Can you work these out from the model? Positions are in its coordinate system, mm. A direction names the side the tool comes from. Give positions to 0.01 mm unless a question says otherwise; leave off trailing zeros. Order: outer loops, then holes, each group sorted by start corner. A loop starts at its lowest first (then second) coordinate and runs counter-clockwise, first axis right, second up. Notation, with made-up numbers: (10, 43.25) - (61, 43.25) arc R8 ccw to (61, 50.25) - close; hole circle Ø11 at (0.25, -20.5). An arc over 180 degrees is marked (long way). Answer as CSV lines item,"result".
```python
from build123d import *

# Parameters (mm, degrees)
SKETCH1_R           = 25
BOSS_EXTRUDE1_DEPTH = 42
CHAMFER1_SIZE       = 1.5


with BuildPart() as part:
    # Sketch1 → Boss-Extrude1 (new body)
    with BuildSketch(Plane(origin=(0, 0, 0), x_dir=(1, 0, 0), z_dir=(0, 1, 0))):
        with Locations(Location((0, 0, 0), (0, 0, 90))):
            Circle(SKETCH1_R)
        with BuildLine():
            ThreePointArc((10, 0), (8.062257748, -5.916079783), (3, -9.539392014))
            Line((3, -9.539392014), (3, -12.8))
            Line((3, -12.8), (-3, -12.8))
            Line((-3, -12.8), (-3, -9.539392014))
            ThreePointArc((-3, -9.539392014), (-5.916079783, 8.062257748), (10, 0))
        make_face(mode=Mode.SUBTRACT)
    extrude(amount=BOSS_EXTRUDE1_DEPTH)

    # Chamfer1
    chamfer1_edges = [part.edges().sort_by_distance(p)[0] for p in [
        (-5.916079783, 42, -8.062257748),
        (-5.916079783, 0, -8.062257748),
    ]]
    chamfer(chamfer1_edges, length=CHAMFER1_SIZE)


solid = part.part
```
1) I want a section at B-B on y = 30. Write out the boundary of the cut face in (x, z).
Answer block:
outline,"circle Ø50 at (0, 0); hole (-3, 9.54) arc R10 ccw (long way) to (3, 9.54) - (3, 12.8) - (-3, 12.8) - close"
2) I'm going to push flat-ended pins straight in: P1, Ø3, axis at x = 8.5, y = 20.5, coming from the -Z side; P2, Ø4, axis at x = -19, y = 28.5, coming from the +Z side; P3, Ø5, axis at x = -1.5, y = 33.5, coming from the +Z side; P4, Ø10, axis at y = 22, z = 4, coming from the +X side. Where does each tip first touch, or does it pass through?
Answer block:
P1,"z = -24"
P2,"z = 18.33"
P3,"z = 25"
P4,"x = 25"
3) Which directions (+Z, -Z, +X, -X, +Y, -Y) give clear straight access to the entire face, cutting with the end or side of a thin tool? Please do faces 1 (the flat face through (-3, 21, 11)), 2 (the flat face through (11, 0, -5)).
Answer block:
face 1,"+Y, -Y"
face 2,"+Z, -Z, +X, -X, -Y"
4) I want a section at D-D on x = 21. Write out the boundary of the cut face in (y, z), plus the area to 3 significant figures.
Answer block:
outline,"(0, -13.56) - (42, -13.56) - (42, 13.56) - (0, 13.56) - close"
area,"1,140 mm2"
5) I want a section at C-C on z = -20. Write out the boundary of the cut face in (x, y).
Answer block:
outline,"(-15, 0) - (15, 0) - (15, 42) - (-15, 42) - close"
6) If we mould it in two halves opening along X, with no side actions, what happens to faces 3 (the cylindrical face through (-7.509, 20.706, -23.846)), 4 (the flat face through (3, 21, 11)), 5 (the flat face through (11, 42, -5))? For each: +X half, -X half, draft (parallel to the pull), parting line (faces both ways), or undercut.
Answer block:
face 3,"parting line"
face 4,"undercut"
face 5,"draft"
7) I need wall thicknesses on line 1 along X through (y, z) = (31, 0); line 2 along X through (y, z) = (19.5, 8); line 3 along Z through (x, y) = (8.5, 40). Which ranges of each line are inside material? Lowest first, please. Write a range as [from, to].
Answer block:
line 1,"[-25, -10], [10, 25]"
line 2,"[-23.69, -6], [6, 23.69]"
line 3,"[-23.51, -5.27], [5.27, 23.51]"
8) I want a section at A-A on x = 0. Write out the boundary of the cut face in (y, z).
Answer block:
outline,"(0, -25) - (42, -25) - (42, -11.5) - (40.5, -10) - (1.5, -10) - (0, -11.5) - close; (0, 12.8) - (42, 12.8) - (42, 25) - (0, 25) - close"
